from build123d import *

# Parameters (mm, degrees)
SKETCH_2_W                  = 74
SKETCH_2_H                  = 35
SKETCH_2_W_2                = 57
SKETCH_2_H_2                = 25
SKETCH_11_W                 = 77
SKETCH_11_H                 = 35
SKETCH_11_W_2               = 57
SKETCH_11_H_2               = 25
EXTRUDE_1_DEPTH             = 22
SKETCH_12_W                 = 23.011901601
SKETCH_12_H                 = 57
CUT_EXTRUDE_9_DEPTH         = 1073.864623333
HOLE_WIZARD_5_5_5_5_1_D     = 5.5
SKETCH_15_W                 = 77
SKETCH_15_H                 = 35
SKETCH_15_W_2               = 57
SKETCH_15_H_2               = 25
EXTRUDE_2_DEPTH             = 22
SKETCH_16_W                 = 45.795478168
SKETCH_16_H                 = 57
CUT_EXTRUDE_10_DEPTH        = 49
HOLE_WIZARD_5_5_5_5_2_D     = 5.5
HOLE_WIZARD_5_5_5_5_2_DEPTH = 50
HOLE_WIZARD_5_5_5_5_2_TIP   = 1.652366702


with BuildPart() as part:
    # 扫描1: sweep along a path in 草图1
    with BuildLine(Plane.XY) as sweep_1_path:
        Line((0, 0), (-1000, 0))
        ThreePointArc((-1000, 0), (-1050, 50), (-1000, 100))
        Line((-1000, 100), (-950, 100))
    # 草图2 → 扫描1 (sweep)
    with BuildSketch(Plane(origin=(0, 0, 0), x_dir=(0, 0, -1), z_dir=(1, 0, 0))):
        Rectangle(SKETCH_2_W, SKETCH_2_H)
        Rectangle(SKETCH_2_W_2, SKETCH_2_H_2, mode=Mode.SUBTRACT)
    sweep(path=sweep_1_path.line)

    # 草图11 → 凸台-拉伸1 (add)
    with BuildSketch(Plane(origin=(0, 0, 0), x_dir=(0, 0, -1), z_dir=(1, 0, 0))):
        Rectangle(SKETCH_11_W, SKETCH_11_H)
        Rectangle(SKETCH_11_W_2, SKETCH_11_H_2, mode=Mode.SUBTRACT)
    extrude(amount=EXTRUDE_1_DEPTH)

    # 草图12 → 切除-拉伸9 (cut, through all)
    with BuildSketch(Plane(origin=(0, 17.5, 0), x_dir=(1, 0, 0), z_dir=(0, 1, 0))):
        with Locations((11.505950801, 0)):
            Rectangle(SKETCH_12_W, SKETCH_12_H)
    extrude(amount=-CUT_EXTRUDE_9_DEPTH, mode=Mode.SUBTRACT)

    # Ø5.5 (5.5) 直径孔1 (through all)
    with Locations(Plane(origin=(0, 17.5, 0), x_dir=(1, 0, 0), z_dir=(0, 1, 0))):
        with Locations((12, 33.5), (12, -33.5)):
            Hole(HOLE_WIZARD_5_5_5_5_1_D / 2)

    # 草图15 → 凸台-拉伸2 (add)
    with BuildSketch(Plane(origin=(-950, 0, 0), x_dir=(0, 0, -1), z_dir=(1, 0, 0))):
        with Locations((0, 100)):
            Rectangle(SKETCH_15_W, SKETCH_15_H)
        with Locations((0, 100)):
            Rectangle(SKETCH_15_W_2, SKETCH_15_H_2, mode=Mode.SUBTRACT)
    extrude(amount=EXTRUDE_2_DEPTH)

    # 草图16 → 切除-拉伸10 (cut)
    with BuildSketch(Plane(origin=(0, 117.5, 0), x_dir=(1, 0, 0), z_dir=(0, 1, 0))):
        with Locations((-927.102260916, 0)):
            Rectangle(SKETCH_16_W, SKETCH_16_H)
    extrude(amount=-CUT_EXTRUDE_10_DEPTH, mode=Mode.SUBTRACT)

    # Ø5.5 (5.5) 直径孔2
    with Locations(Plane(origin=(0, 117.5, 0), x_dir=(1, 0, 0), z_dir=(0, 1, 0))):
        with Locations((-938, 33.5), (-938, -33.5)):
            Hole(HOLE_WIZARD_5_5_5_5_2_D / 2, depth=HOLE_WIZARD_5_5_5_5_2_DEPTH)
            with Locations((0, 0, -(HOLE_WIZARD_5_5_5_5_2_DEPTH + HOLE_WIZARD_5_5_5_5_2_TIP / 2))):  # 118° drill point
                Cone(0, HOLE_WIZARD_5_5_5_5_2_D / 2, HOLE_WIZARD_5_5_5_5_2_TIP, mode=Mode.SUBTRACT)


solid = part.part
Geometry: final body of the model. Coordinates: model frame, mm. A direction names the side the tool comes from. Round coordinates to 2 decimals unless told otherwise and drop trailing zeros. Order: outer loops, then holes, each group sorted by start corner. A loop starts at its lowest first (then second) coordinate and runs counter-clockwise, first axis right, second up. Notation, with made-up numbers: (56, 31.25) - (62, 31.25) arc R20 cw to (62, 65.25) - close; hole circle Ø7 at (2, 24). An arc over 180 degrees is marked (long way). Write each question's results on one line, items separated by ' | '.
Item 1: Reachability of faces 1 (the flat face through (11, 0, 38.5)), 2 (the flat face through (-507, -12.5, 0)), 3 (the flat face through (-973, 82.5, 1)) from +Z, -Z, +X, -X, +Y, -Y: full face, straight path, thin tool, end or side. Return the list, or none.
Completed:
face 1: +Z, +X, -X, +Y, -Y | face 2: +X | face 3: +Z, -Z, +X
Item 2: Mould query, pull axis X, two halves, no side actions, for faces 4 (the cylindrical face through (-1037.49, 49.18, -0.4)), 5 (the flat face through (-496, -17.5, 1)), 6 (the cylindrical face through (-1062.485, 48.626, 0.399)), 7 (the cylindrical face through (-1067.484, 48.516, -0.518)). Classes: pulls with the +X half, pulls with the -X half, needs draft (parallel to the pull), parting line crosses it, or undercut.
Completed:
face 4: undercut | face 5: needs draft | face 6: undercut | face 7: pulls with the -X half
Item 3: Section D-D, the plane y = 0.5. Return the cut outline in (x, z).
Completed:
outline: (-1045.89, -37) - (0, -37) - (0, -38.5) - (22, -38.5) - (22, -28.5) - (-1038.16, -28.5) - (-1038.16, 28.5) - (22, 28.5) - (22, 38.5) - (0, 38.5) - (0, 37) - (-1045.89, 37) - close; hole circle Ø5.5 at (12, -33.5); hole circle Ø5.5 at (12, 33.5)
Item 4: First-contact query: pin 1 Ø5 at (x, y) = (-894, 18.5) entering from -Z; pin 2 Ø4 at (x, y) = (-153.5, 1.5) entering from +Z; pin 3 Ø10 at (y, z) = (48, -24.5) entering from -X; pin 4 Ø5 at (x, z) = (12, -33.5) entering from -Y. Flat tips, straight axial feed; report the tip coordinate or a pass-through.
Completed:
pin 1: z = -37 | pin 2: z = 37 | pin 3: x = -1067.5 | pin 4: through
Item 5: Section B-B, the plane x = -368.5. Return the cut outline in (y, z).
Completed:
outline: (-17.5, -37) - (17.5, -37) - (17.5, 37) - (-17.5, 37) - close; hole (-12.5, -28.5) - (12.5, -28.5) - (12.5, 28.5) - (-12.5, 28.5) - close
Item 6: Material intervals for line 1 along Z through (x, y) = (12, 9.5); line 2 along Y through (x, z) = (-964, -6.5); line 3 along Y through (x, z) = (-269, -15.5), sorted ascending. Write a range as [from, to].
Completed:
line 1: [-38.5, -36.25], [-30.75, -28.5], [28.5, 30.75], [36.25, 38.5] | line 2: [-17.5, -12.5], [12.5, 17.5], [82.5, 87.5], [112.5, 117.5] | line 3: [-17.5, -12.5], [12.5, 17.5]
Item 7: Section A-A, the plane z = -12. Return the cut outline in (x, y).
Completed:
outline: (-1000, -17.5) - (0, -17.5) - (0, -12.5) - (-1000, -12.5) arc R62.5 cw to (-1000, 112.5) - (-950, 112.5) - (-950, 117.5) - (-1000, 117.5) arc R67.5 ccw to start; (-1000, 12.5) - (0, 12.5) - (0, 17.5) - (-1000, 17.5) arc R32.5 cw to (-1000, 82.5) - (-950, 82.5) - (-950, 87.5) - (-1000, 87.5) arc R37.5 ccw to start
Item 8: Section C-C, the plane y = 62. Return the cut outline in (x, z), and give its area (3 significant figures).
Completed:
outline: (-1066.42, -37) - (-1030.2, -37) - (-1030.2, 37) - (-1066.42, 37) - close; hole (-1061.34, -28.5) - (-1035.53, -28.5) - (-1035.53, 28.5) - (-1061.34, 28.5) - close | area: 1,210 mm^2
